Could you check a few things on this model? Use its own coordinates, in mm. A direction names the side the tool comes from. Give positions to 0.01 mm unless a question says otherwise; leave off trailing zeros. Order: outer loops, then holes, each group sorted by start corner. A loop starts at its lowest first (then second) coordinate and runs counter-clockwise, first axis right, second up. Notation, with made-up numbers: (-7, 36) -> (31, 36) arc R23 ccw to (31, 60) -> close; hole circle Ø10 at (80, 66.25). An arc over 180 degrees is marked (long way). Write each question's results on one line, items separated by ' | '.
```python
from build123d import *

# Parameters (mm, degrees)
SKETCH1_R             = 45
SKETCH1_R_2           = 25
BOSS_EXTRUDE1_DEPTH   = 12
SKETCH2_R             = 40
SKETCH2_R_2           = 25
BOSS_EXTRUDE2_DEPTH   = 3
M4_TAPPED_HOLE2_D     = 3.3
M4_TAPPED_HOLE2_DEPTH = 10.1
M4_TAPPED_HOLE2_TIP   = 0.991420021


with BuildPart() as part:
    # Sketch1 → Boss-Extrude1 (new body)
    with BuildSketch(Plane.XY):
        Circle(SKETCH1_R)
        Circle(SKETCH1_R_2, mode=Mode.SUBTRACT)
    extrude(amount=BOSS_EXTRUDE1_DEPTH)

    # Sketch2 → Boss-Extrude2 (add)
    with BuildSketch(Plane.XY.offset(12)):
        Circle(SKETCH2_R)
        Circle(SKETCH2_R_2, mode=Mode.SUBTRACT)
    extrude(amount=BOSS_EXTRUDE2_DEPTH)

    # M4 Tapped Hole2
    with Locations(Plane(origin=(32.04293994, 18.5, 0), x_dir=(-1, 0, 0), z_dir=(0, 0, -1))):
        with Locations((0, 0), (32.04293994, 18.5), (64.08587988, 0), (64.08587988, -37), (32.04293994, -55.5), (0, -37)):
            Hole(M4_TAPPED_HOLE2_D / 2, depth=M4_TAPPED_HOLE2_DEPTH)
            with Locations((0, 0, -(M4_TAPPED_HOLE2_DEPTH + M4_TAPPED_HOLE2_TIP / 2))):  # 118° drill point
                Cone(0, M4_TAPPED_HOLE2_D / 2, M4_TAPPED_HOLE2_TIP, mode=Mode.SUBTRACT)


solid = part.part
```
Q1. Thinking about a two-plate mould opening in Y: for faces 1 (the cylindrical face through (20.765, -39.923, 5.916)), 2 (the cylindrical face through (-33.69, -18.43, 5.12)), 3 (the flat face through (17.22, 18.34, 15)), which applies, +Y half, -Y half, draft (parallel to the pull), parting line (faces both ways), or undercut?
Here are the results:
face 1: parting line | face 2: undercut | face 3: draft
Q2. Suppose I cut it at B-B on z = 8. Please give me the cut outline in (x, y).
Here are the results:
outline: circle Ø90 at (0, 0); hole circle Ø3.3 at (-32.04, -18.5); hole circle Ø3.3 at (-32.04, 18.5); hole circle Ø50 at (0, 0); hole circle Ø3.3 at (0, -37); hole circle Ø3.3 at (0, 37); hole circle Ø3.3 at (32.04, -18.5); hole circle Ø3.3 at (32.04, 18.5)
Q3. I need wall thicknesses on line 1 along Y through (x, z) = (0, 2.75); line 2 along X through (y, z) = (-1, 8); line 3 along X through (y, z) = (18.5, 4.25). Which ranges of each line are inside material? Lowest first, please.
Here are the results:
line 1: y = -45 to -38.65, -35.35 to -25, 25 to 35.35, 38.65 to 45 | line 2: x = -44.99 to -24.98, 24.98 to 44.99 | line 3: x = -41.02 to -33.69, -30.39 to -16.82, 16.82 to 30.39, 33.69 to 41.02
Q4. I'm going to push flat-ended pins straight in: pin 1 Ø5 at (y, z) = (21.5, 5) entering from +X; pin 2 Ø1.5 at (y, z) = (30, 12.5) entering from -X; pin 3 Ø3 at (y, z) = (21, 7.5) entering from -X. Where does each tip first touch, or does it pass through?
Here are the results:
pin 1: stops at x = 40.79 | pin 2: stops at x = -34.03 | pin 3: stops at x = -40.56
Q5. Suppose I cut it at A-A on y = 0. Please give me the cut outline in (x, z).
Here are the results:
outline: (-45, 0) -> (-25, 0) -> (-25, 15) -> (-40, 15) -> (-40, 12) -> (-45, 12) -> close; (25, 0) -> (45, 0) -> (45, 12) -> (40, 12) -> (40, 15) -> (25, 15) -> close
Q6. Suppose I cut it at C-C on x = -23.5. Please give me the cut outline in (y, z).
Here are the results:
outline: (-38.38, 0) -> (-8.53, 0) -> (-8.53, 15) -> (-32.37, 15) -> (-32.37, 12) -> (-38.38, 12) -> close; (8.53, 0) -> (38.38, 0) -> (38.38, 12) -> (32.37, 12) -> (32.37, 15) -> (8.53, 15) -> close
Q7. Suppose I cut it at D-D on y = -31. Please give me the cut outline in (x, z), and give its area (3 significant figures).
Here are the results:
outline: (-32.62, 0) -> (32.62, 0) -> (32.62, 12) -> (25.28, 12) -> (25.28, 15) -> (-25.28, 15) -> (-25.28, 12) -> (-32.62, 12) -> close | area: 935 mm²
Q8. For faces 4 (the cylindrical face through (-33.69, 18.57, 5.12)), 5 (the cylindrical face through (-8.67, -39.05, 13.48)), 6 (the flat face through (19, -19, 0)), which set-ups out of +Z, -Z, +X, -X, +Y, -Y let a thin tool reach every point of the face, with its end or its side?
Here are the results:
face 4: -Z | face 5: +Z | face 6: -Z, +X, -X, +Y, -Y
